The listing builds one solid part. Answer for the finished solid, in the listing's coordinates (mm). Face numbers are marked on the shaded views. A direction names the side the tool comes from. Round coordinates to 2 decimals unless told otherwise and drop trailing zeros. Write each loop counter-clockwise with the first axis right and the second up, starting at its lowest first coordinate (ties: lowest second). Pieces come first, ordered by that corner, then holes. Notation, with made-up numbers: (29.25, 66) - (52.25, 66) arc R30 ccw to (52.25, 105) - close; hole circle Ø4 at (32.25, -18). An arc over 180 degrees is marked (long way). Return JSON: item names as keys, results as strings. Group by question number.
(1) Determine the mould class of the marked faces 6, 7, 8 and 9 for opening direction X: +X half, -X half, draft (parallel to the pull), parting line (faces both ways), or undercut.
(2) Section A-A, the plane x = 0 is taken. Write down the section's boundary in (y, z).
(3) Section C-C, the plane x = -2.75 is taken. Write down the section's boundary in (y, z), then the cut area to 3 significant figures.
(4) Which of the six approach directions +Z, -Z, +X, -X, +Y, -Y give full straight-line access (tool end or side, diameter ignored) to the marked faces 1, 2, 3, 4 and 5?
(5) This flat-tipped pin is pushed along its axis until it touches: pin 1 (2 mm diameter, centred on y = 6.5, z = -0.5, fed in from +X). Where does it stop, or does it pass through?
(6) Find the intervals of material crossed by line 1 along Z through (x, y) = (0, 3.5); line 2 along Z through (x, y) = (0, 10); line 3 along Y through (x, z) = (-3, -1.5), in increasing order. Write a range as [from, to].
(7) Section B-B, the plane y = -5.25 is taken. Write down the section's boundary in (x, z), then the cut area to 3 significant figures.
(8) Section D-D, the plane z = -2.75 is taken. Write down the section's boundary in (x, y), then the cut area to 3 significant figures.
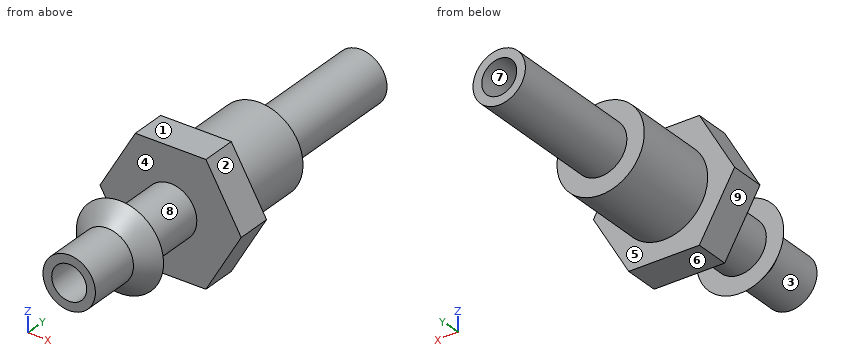
```python
from build123d import *

# Parameters (mm, degrees)
HEX_7AF_DEPTH     = 2
BORE_PROFILE_2_R  = 1
FUEL_BORE_2_DEPTH = 24.613202522


with BuildPart() as part:
    # Lower Spigot Profile → Lower Spigot and Collar (revolve)
    with BuildSketch(Plane.XY, mode=Mode.PRIVATE) as lower_spigot_and_collar_sk:
        Polygon((0, 0), (0, -8), (1.5, -8), (1.5, -5), (2.5, -4), (1.5, -4), (1.5, 0), align=None)
    revolve(lower_spigot_and_collar_sk.sketch.rotate(Axis((0, 0, 0), (0, -1, 0)), 90), axis=Axis((0, 0, 0), (0, -1, 0)))

    # Hex Profile 7AF → Hex 7AF (add)
    with BuildSketch(Plane(origin=(0, 0, 0), x_dir=(1, 0, 0), z_dir=(0, 1, 0))):
        Polygon((4.041451884, 0), (2.020725942, 3.5), (-2.020725942, 3.5), (-4.041451884, 0), (-2.020725942, -3.5), (2.020725942, -3.5), align=None)
    extrude(amount=HEX_7AF_DEPTH)

    # Upper Pipe Profile → Upper Pipe (revolve)
    with BuildSketch(Plane.XY):
        Polygon((0, 2), (0, 15), (1.5, 15), (1.5, 7), (2.5, 7), (2.5, 2), align=None)
    revolve(axis=Axis((0, 2, 0), (0, 1, 0)))

    # Bore Profile Ø2 → Fuel Bore Ø2 (cut, through all)
    with BuildSketch(Plane(origin=(0, 15, 0), x_dir=(1, 0, 0), z_dir=(0, 1, 0))):
        with Locations(Location((0, 0, 0), (0, 0, 180))):
            Circle(BORE_PROFILE_2_R)
    extrude(amount=-FUEL_BORE_2_DEPTH, mode=Mode.SUBTRACT)


solid = part.part
```
Working result:
{
 "1": {"face 6": "draft", "face 7": "undercut", "face 8": "parting line", "face 9": "-X half"},
 "2": {"outline": "(-8, -1.5) - (-5, -1.5) - (-4, -2.5) - (-4, -1.5) - (0, -1.5) - (0, -3.5) - (2, -3.5) - (2, -2.5) - (7, -2.5) - (7, -1.5) - (15, -1.5) - (15, -1) - (-8, -1) - close; (-8, 1) - (15, 1) - (15, 1.5) - (7, 1.5) - (7, 2.5) - (2, 2.5) - (2, 3.5) - (0, 3.5) - (0, 1.5) - (-4, 1.5) - (-4, 2.5) - (-5, 1.5) - (-8, 1.5) - close"},
 "3": {"outline": "(0, -2.24) - (2, -2.24) - (2, 2.24) - (0, 2.24) - close", "area": "8.95 mm^2"},
 "4": {"face 1": "+Z, +X, -X, +Y, -Y", "face 2": "+Z, +X, +Y, -Y", "face 3": "-Y", "face 4": "none", "face 5": "+Y"},
 "5": {"pin 1": "stops at x = 2.5"},
 "6": {"line 1": "z = [-2.5, -1], [1, 2.5]", "line 2": "z = [-1.5, -1], [1, 1.5]", "line 3": "y = [0, 2]"},
 "7": {"outline": "circle Ø3 at (0, 0); hole circle Ø2 at (0, 0)", "area": "3.93 mm^2"},
 "8": {"outline": "(-2.45, 0) - (2.45, 0) - (2.45, 2) - (-2.45, 2) - close", "area": "9.81 mm^2"}
}
